Part model, mm, in its own coordinate system. A direction names the side the tool comes from. Coordinates: 2 decimals unless noted, no trailing zeros. Loops run counter-clockwise (first coordinate to the right, second up) from the corner with the lowest first, then second, coordinate; pieces in that order, holes last. Notation, with made-up numbers: (-34.75, 10) - (10.25, 10) arc R14 ccw to (10.25, 16) - close; hole circle Ø5 at (87.25, -10). An arc over 180 degrees is marked (long way). Use a Markdown table: item, result. Add a question column.
1. Band-saw the part on D-D, the plane y = -8. Give the cut face in (x, z).
2. 3-axis set-ups, long thin cutter, end or side, ignore diameter. For faces 1 (the flat face through (-1, 5, 0)), 2 (the flat face through (-14.545, -6, 10)): which of +Z, -Z, +X, -X, +Y, -Y reach the whole face in a straight line?
3. Drop flat-ended pins along their axis: pin 1 (6 mm diameter, centred on x = 3, z = 11, fed in from -Y); pin 2 (7.5 mm diameter, centred on x = -1, y = -8.5, fed in from -Z). Give the stop position or say it passes through.
4. Wall check: probe 1 along X at (y, z) = (0.75, 25); probe 2 along X at (y, z) = (-9.5, 6.5); probe 3 along X at (y, z) = (-5, 28.5). Give the ranges that are in metal, low to high. Write a range as [from, to].
5. Pull direction Z, two halves, no side cores. Call faces 3 (the cylindrical face through (16.237, 1.317, 3.846)), 4 (the flat face through (-1, 16.527, 15)), 5 (the flat face through (0, -6, 20)): pulls with the +Z half, pulls with the -Z half, needs draft (parallel to the pull), parting line crosses it, or undercut.
6. Band-saw the part on B-B, the plane z = 10.5. Give the cut face in (x, y), plus the area to 3 significant figures.
7. Band-saw the part on A-A, the plane z = 25. Give the cut face in (x, y), plus the area to 3 significant figures.
8. Band-saw the part on C-C, the plane z = 5. Give the cut face in (x, y), plus the area to 3 significant figures.
from build123d import *

# Parameters (mm, degrees)
SKETCH_1_W          = 48
SKETCH_1_H          = 30
EXTRUDE_1_DEPTH     = 30
SKETCH_2_W          = 28
SKETCH_2_H          = 15
CUT_EXTRUDE_1_DEPTH = 20
SKETCH_3_R          = 2.2
CUT_EXTRUDE_2_DEPTH = 20
SKETCH_4_R          = 2.5
CUT_EXTRUDE_3_DEPTH = 30


with BuildPart() as part:
    # 草图1 → 凸台-拉伸1 (new body)
    with BuildSketch(Plane.XY):
        with Locations((-0.545454545, 1.527272727)):
            Rectangle(SKETCH_1_W, SKETCH_1_H)
    extrude(amount=EXTRUDE_1_DEPTH)

    # 草图2 → 切除-拉伸1 (cut)
    with BuildSketch(Plane(origin=(0, 0, 0), x_dir=(-1, 0, 0), z_dir=(0, 0, -1))):
        with Locations((0.545454545, -5.972727273)):
            Rectangle(SKETCH_2_W, SKETCH_2_H)
    extrude(amount=-CUT_EXTRUDE_1_DEPTH, mode=Mode.SUBTRACT)

    # 草图3 → 切除-拉伸2 (cut)
    with BuildSketch(Plane(origin=(0, 0, 20), x_dir=(-1, 0, 0), z_dir=(0, 0, -1))):
        with Locations((-10.454545455, -3.472727273)):
            Circle(SKETCH_3_R)
        with Locations((11.545454545, -3.472727273)):
            Circle(SKETCH_3_R)
    extrude(amount=-CUT_EXTRUDE_2_DEPTH, mode=Mode.SUBTRACT)

    # 草图4 → 切除-拉伸3 (cut)
    with BuildSketch(Plane.XZ.offset(13.472727273)):
        with Locations(Location((-19.545454545, 5, 0), (0, 0, 270))):
            Circle(SKETCH_4_R)
        with Locations(Location((-19.545454545, 25, 0), (0, 0, 270))):
            Circle(SKETCH_4_R)
        with Locations(Location((18.454545455, 25, 0), (0, 0, 270))):
            Circle(SKETCH_4_R)
        with Locations(Location((18.454545455, 5, 0), (0, 0, 270))):
            Circle(SKETCH_4_R)
    extrude(amount=-CUT_EXTRUDE_3_DEPTH, mode=Mode.SUBTRACT)


solid = part.part
Geometry check:
| question | item | result |
|---|---|---|
| 1 | outline | (-24.55, 0) - (-14.55, 0) - (-14.55, 20) - (13.45, 20) - (13.45, 0) - (23.45, 0) - (23.45, 30) - (-24.55, 30) - close; hole circle Ø5 at (-19.55, 5); hole circle Ø5 at (-19.55, 25); hole circle Ø5 at (18.45, 5); hole circle Ø5 at (18.45, 25) |
| 2 | face 1 | -Z, +X, -X, +Y, -Y |
| 2 | face 2 | -Z, -Y |
| 3 | pin 1 | stops at y = 1.53 |
| 3 | pin 2 | stops at z = 20 |
| 4 | probe 1 | x = [-24.55, -22.05], [-17.05, 15.95], [20.95, 23.45] |
| 4 | probe 2 | x = [-24.55, -21.55], [-17.55, -14.55], [13.45, 16.45], [20.45, 23.45] |
| 4 | probe 3 | x = [-24.55, -13.13], [-9.96, 8.87], [12.04, 23.45] |
| 5 | face 3 | undercut |
| 5 | face 4 | needs draft |
| 5 | face 5 | pulls with the -Z half |
| 6 | outline | (-24.55, -13.47) - (-14.55, -13.47) - (-14.55, 1.53) - (13.45, 1.53) - (13.45, -13.47) - (23.45, -13.47) - (23.45, 16.53) - (-24.55, 16.53) - close |
| 6 | area | 1,020 mm^2 |
| 7 | outline | (-24.55, -13.47) - (-22.05, -13.47) - (-22.05, 16.53) - (-24.55, 16.53) - close; (-17.05, -13.47) - (15.95, -13.47) - (15.95, 16.53) - (-17.05, 16.53) - close; (20.95, -13.47) - (23.45, -13.47) - (23.45, 16.53) - (20.95, 16.53) - close; hole circle Ø4.4 at (-11.55, -3.47); hole circle Ø4.4 at (10.45, -3.47) |
| 7 | area | 1,110 mm^2 |
| 8 | outline | (-24.55, -13.47) - (-22.05, -13.47) - (-22.05, 16.53) - (-24.55, 16.53) - close; (-17.05, -13.47) - (-14.55, -13.47) - (-14.55, 1.53) - (13.45, 1.53) - (13.45, -13.47) - (15.95, -13.47) - (15.95, 16.53) - (-17.05, 16.53) - close; (20.95, -13.47) - (23.45, -13.47) - (23.45, 16.53) - (20.95, 16.53) - close |
| 8 | area | 720 mm^2 |
